```python
from build123d import *

# Parameters (mm, degrees)
EXTRUDE_405_DEPTH        = 7.5
FILLET_1252_R            = 0.6
SKETCH_7_R               = 1.6
CUT_EXTRUDE_1_DEPTH      = 761.624250205
PATTERN_CIRCULAR_1_COUNT = 2
PATTERN_CIRCULAR_1_ANGLE = 60


with BuildPart() as part:
    # 草图1 → Extrude 405 (new body)
    with BuildSketch(Plane(origin=(0, 0, 0), x_dir=(0, 0, -1), z_dir=(1, 0, 0))):
        Polygon((9, 5.196152423), (9, -5.196152423), (0, -10.392304845), (-9, -5.196152423), (-9, 5.196152423), (0, 10.392304845), align=None)
    extrude(amount=EXTRUDE_405_DEPTH)

    # 草图2 → 凸台-旋转1 (revolve)
    with BuildSketch(Plane.XY, mode=Mode.PRIVATE) as revolve_1_sk:
        Polygon((0, 0), (760.5, 0), (760.5, 4.4845), (760.5, 6), (730.5, 6), (0, 6), align=None)
    revolve(revolve_1_sk.sketch.rotate(Axis((0, 0, 0), (1, 0, 0)), 90), axis=Axis((0, 0, 0), (1, 0, 0)))

    # 草图3 → 切除-旋转1 (revolve, cut)
    with BuildSketch(Plane.XY):
        Polygon((0, 9), (3.690598923, 15.392304845), (3.690598923, 20.392304845), (-10, 20.392304845), (-10, 9), align=None)
    revolve(axis=Axis((0, 0, 0), (1, 0, 0)), mode=Mode.SUBTRACT)

    # 草图5 → 切除-旋转5 (revolve, cut)
    with BuildSketch(Plane.XY, mode=Mode.PRIVATE) as cut_revolve_5_sk:
        Polygon((7.5, 8.315), (6.9, 8.661410162), (6.9, 10.392304845), (7.5, 10.392304845), align=None)
    revolve(cut_revolve_5_sk.sketch.rotate(Axis((0, 0, 0), (1, 0, 0)), 180), axis=Axis((0, 0, 0), (1, 0, 0)), mode=Mode.SUBTRACT)

    # Fillet 1252
    fillet_1252_edges = [part.edges().sort_by_distance(p)[0] for p in [
        (7.5, 0, -6),
    ]]
    fillet(fillet_1252_edges, radius=FILLET_1252_R)

    # 草图6 → 切除-旋转4 (revolve, cut)
    with BuildSketch(Plane.XY, mode=Mode.PRIVATE) as cut_revolve_4_sk:
        Polygon((759.625, 6), (761.375, 6), (760.5, 4.484455543), align=None)
    revolve(cut_revolve_4_sk.sketch.rotate(Axis((0, 0, 0), (1, 0, 0)), 90), axis=Axis((0, 0, 0), (1, 0, 0)), mode=Mode.SUBTRACT)

    # 草图7 → 切除-拉伸1 (cut, symmetric)
    with BuildSketch(Plane.XY):
        with Locations((3.8, 0)):
            Circle(SKETCH_7_R)
    cut_extrude_1 = extrude(amount=CUT_EXTRUDE_1_DEPTH, both=True, mode=Mode.SUBTRACT)

    # 阵列(圆周)1: 切除-拉伸1 ×2 about axis
    pattern_circular_1_axis = Axis((0, 0, 0), (1, 0, 0))
    for i in range(1, PATTERN_CIRCULAR_1_COUNT):
        add(cut_extrude_1.rotate(pattern_circular_1_axis, i * PATTERN_CIRCULAR_1_ANGLE / (PATTERN_CIRCULAR_1_COUNT - 1)), mode=Mode.SUBTRACT)


solid = part.part
```
Part model, mm, in its own coordinate system. A direction names the side the tool comes from. Round coordinates to 2 decimals unless told otherwise and drop trailing zeros. Loops run counter-clockwise (first coordinate to the right, second up) from the corner with the lowest first, then second, coordinate; pieces in that order, holes last. Notation, with made-up numbers: (24.25, -33.5) -> (52.25, -33.5) arc R19 cw to (52.25, -6.5) -> close; hole circle Ø11 at (43, 61.5). An arc over 180 degrees is marked (long way). Use one line per item in the form item = value. Start each with the question number.
Item 1: Drill centre lines: line 1 along Y through (x, z) = (3.8, 4.5); line 2 along X through (y, z) = (-3.75, 1.5); line 3 along Z through (x, y) = (133, 4). Where is each one in solid material? Low to high.
Item 2: Band-saw the part on A-A (x = 193.5). List the corners of the cut face in (y, z), plus the area to 3 significant figures.
Item 3: Tool access for faces 1 (the flat face through (6.9, 8.4, -2.7)), 2 (the flat face through (0, 0, 0)): list every direction of +Z, -Z, +X, -X, +Y, -Y with a clear straight run to the whole face (end or side of a thin tool).
Item 4: Drop flat-ended pins along their axis: pin 1 Ø8 at (x, y) = (595.5, 2) entering from +Z; pin 2 Ø1.5 at (x, z) = (217.5, -4) entering from +Y; pin 3 Ø3 at (x, z) = (516, -5) entering from -Y; pin 4 Ø3 at (x, y) = (3.8, 0) entering from +Z. Give the stop position or say it passes through.
Data:
q1.line_1 = -4.59 to -1.6, 1.6 to 7.79
q1.line_2 = 0 to 2.31, 5.29 to 760.5
q1.line_3 = -4.47 to 4.47
q2.outline = circle Ø12 at (0, 0)
q2.area = 113 mm^2
q3.face_1 = +X
q3.face_2 = +Z, -Z, -X, +Y, -Y
q4.pin_1 = 6
q4.pin_2 = 5.04
q4.pin_3 = -4.87
q4.pin_4 = through
